Drawing for the job (mm, zero at the part's lowest x, y, z). A direction names the side the tool comes from. Round coordinates to 2 decimals unless told otherwise and drop trailing zeros. Loops run counter-clockwise (first coordinate to the right, second up) from the corner with the lowest first, then second, coordinate; pieces in that order, holes last. Notation, with made-up numbers: M 73,11.25 L 95,11.25 A21 cw 95,20.25 Z; hole C -16.75,10 d10. An arc over 180 degrees is marked long. Answer in a Markdown table with one row per item.
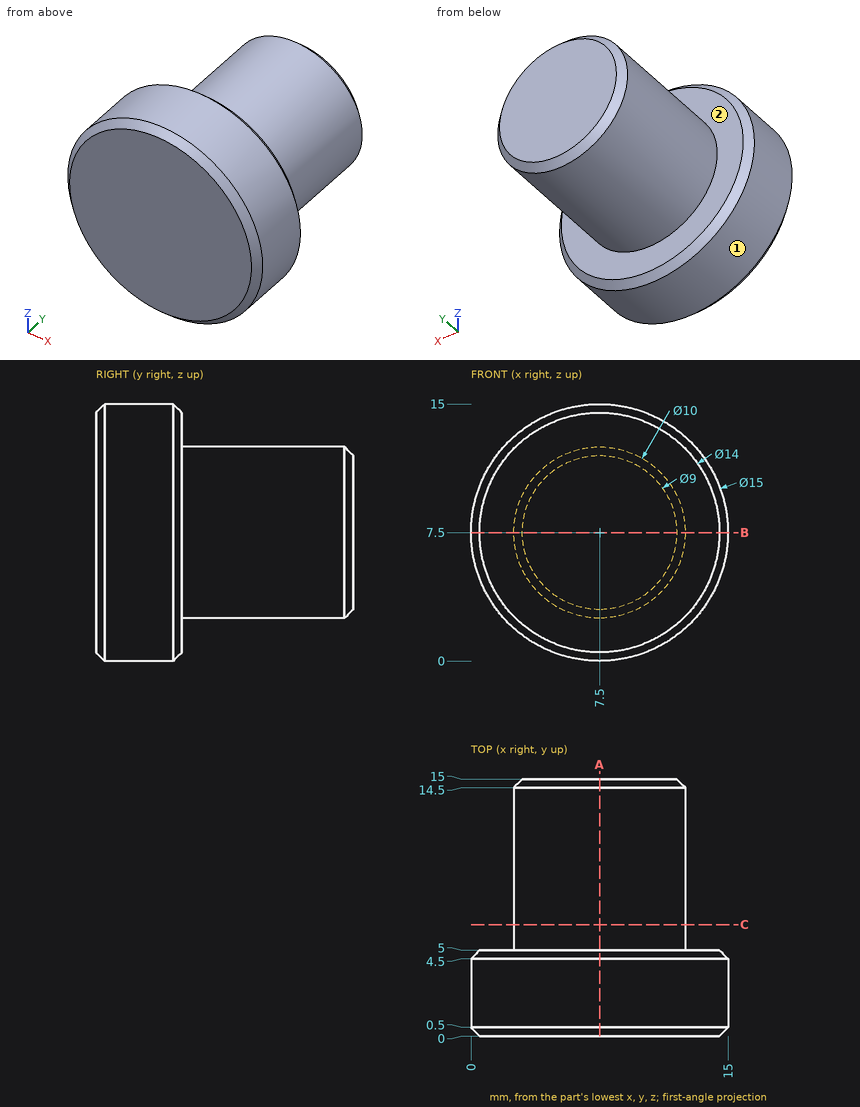
1. Saw through at A-A (x = 7.5). Write the cut outline in (y, z).
Verdict:
| item | result |
|---|---|
| outline | M 0,0.5 L 0.5,0 L 4.5,0 L 5,0.5 L 5,2.5 L 14.5,2.5 L 15,3 L 15,12 L 14.5,12.5 L 5,12.5 L 5,14.5 L 4.5,15 L 0.5,15 L 0,14.5 Z |
2. Tool access for the marked faces 1 and 2: list every direction of +Z, -Z, +X, -X, +Y, -Y with a clear straight run to the whole face (end or side of a thin tool).
Verdict:
| item | result |
|---|---|
| face 1 | +Y, -Y |
| face 2 | +Y |
3. Wall check: probe 1 along Y at (x, z) = (3, 11); probe 2 along X at (y, z) = (12.5, 4.5); probe 3 along Z at (x, y) = (7.25, 9.75). Give the ranges that are in metal, low to high.
Verdict:
| item | result |
|---|---|
| probe 1 | y = 0 to 5 |
| probe 2 | x = 3.5 to 11.5 |
| probe 3 | z = 2.51 to 12.49 |
4. Saw through at C-C (y = 6.5). Write the cut outline in (x, z), and give its area (3 significant figures).
Verdict:
| item | result |
|---|---|
| outline | C 7.5,7.5 d10 |
| area | 78.5 mm² |
5. Saw through at B-B (z = 7.5). Write the cut outline in (x, y), and give its area (3 significant figures).
Verdict:
| item | result |
|---|---|
| outline | M 0,0.5 L 0.5,0 L 14.5,0 L 15,0.5 L 15,4.5 L 14.5,5 L 12.5,5 L 12.5,14.5 L 12,15 L 3,15 L 2.5,14.5 L 2.5,5 L 0.5,5 L 0,4.5 Z |
| area | 174 mm² |
6. Pin check, flat tips, straight feed: pin 1 (6 mm diameter, centred on y = 11, z = 9.5, fed in from -X); pin 2 (1 mm diameter, centred on x = 12.5, y = 7, fed in from +Z); pin 3 (4 mm diameter, centred on y = 2.5, z = 2.5, fed in from -X). Stop position of each tip, or through.
Verdict:
| item | result |
|---|---|
| pin 1 | stops at x = 2.5 |
| pin 2 | stops at z = 9.68 |
| pin 3 | stops at x = 0.63 |
